```python
from build123d import *

# Parameters (mm, degrees)
SKETCH1_W           = 40
SKETCH1_H           = 15
BOSS_EXTRUDE1_DEPTH = 20
SKETCH2_W           = 35.032113562
SKETCH2_H           = 10.660333008
CUT_EXTRUDE1_DEPTH  = 10
SKETCH3_R           = 4
BOSS_EXTRUDE2_DEPTH = 35.032113562
SKETCH4_R           = 3.332307017
BOSS_EXTRUDE3_DEPTH = 10
BOSS_EXTRUDE4_START = 10
SKETCH5_R           = 3.332307017
BOSS_EXTRUDE4_DEPTH = 10
SCALE1_SCALE        = 0.7


with BuildPart() as part:
    # Sketch1 → Boss-Extrude1 (new body)
    with BuildSketch(Plane(origin=(0, 0, 0), x_dir=(1, 0, 0), z_dir=(0, 1, 0))):
        Rectangle(SKETCH1_W, SKETCH1_H)
    extrude(amount=BOSS_EXTRUDE1_DEPTH)

    # Sketch2 → Cut-Extrude1 (cut)
    with BuildSketch(Plane(origin=(0, 20, 0), x_dir=(1, 0, 0), z_dir=(0, 1, 0))):
        Rectangle(SKETCH2_W, SKETCH2_H)
    extrude(amount=-CUT_EXTRUDE1_DEPTH, mode=Mode.SUBTRACT)

    # Sketch3 → Boss-Extrude2 (add)
    with BuildSketch(Plane(origin=(-17.516056781, 0, 0), x_dir=(0, 0, -1), z_dir=(1, 0, 0))):
        with Locations((0, 10)):
            Circle(SKETCH3_R)
    extrude(amount=BOSS_EXTRUDE2_DEPTH)

    # Sketch4 → Boss-Extrude3 (add)
    with BuildSketch(Plane.ZY.offset(20)):
        with Locations((0, 10)):
            Circle(SKETCH4_R)
    extrude(amount=BOSS_EXTRUDE3_DEPTH)

    # Sketch5 → Boss-Extrude4 (add)
    with BuildSketch(Plane(origin=(20, 0, 0), x_dir=(0, 0, -1), z_dir=(1, 0, 0)).offset(BOSS_EXTRUDE4_START)):
        with Locations(Location((0, 10, 0), (0, 0, 180))):
            Circle(SKETCH5_R)
    extrude(amount=-BOSS_EXTRUDE4_DEPTH)


with BuildPart() as part_1:
    # Scale1: scaled about (0, 0, 0)
    add(part.part.scale(SCALE1_SCALE))


solid = part_1.part
```
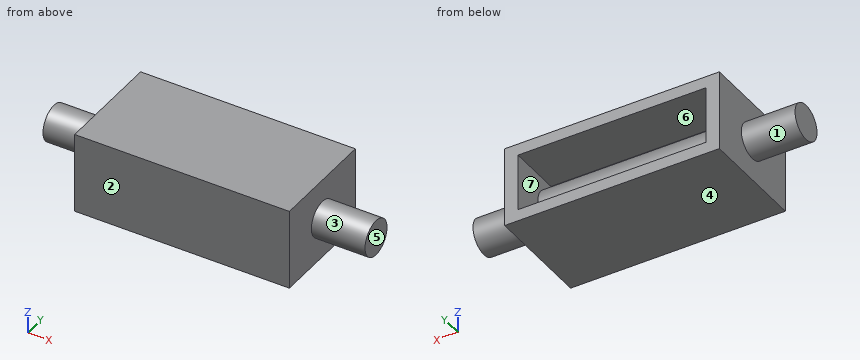
Check sheet for the modelled part. Datum: model origin and axes. Units: mm. Face numbers are marked on the shaded views. A direction names the side the tool comes from. Coordinates: 2 decimals unless noted, no trailing zeros. Order: outer loops, then holes, each group sorted by start corner. A loop starts at its lowest first (then second) coordinate and runs counter-clockwise, first axis right, second up. Notation, with made-up numbers: M 79.5,32.25 L 92.5,32.25 A23 cw 92.5,70.25 Z; hole C -25.75,59.25 d5. An arc over 180 degrees is marked long. One line per question, with ' | ' between items. Start each with the question number.
Item 1: Access from +Z, -Z, +X, -X, +Y, -Y to the whole of each face (thin tool, end or side, straight path). Record for the marked faces 1, 2 and 3.
Item 2: Sectioned sample at A-A on y = 13.25. Record the cut outline in (x, z), and give its area (3 significant figures).
Item 3: Material ranges on line 1 (X direction, y = 12.25, z = 2); line 2 (Z direction, x = -6, y = 10); line 3 (Z direction, x = -4, y = 7.25), recorded low to high.
Item 4: Sectioned sample at D-D on y = 3.25. Record the cut outline in (x, z), and give its area (3 significant figures).
Item 5: Sectioned sample at B-B on z = 0. Record the cut outline in (x, y), and give its area (3 significant figures).
Item 6: Mould release check, pull along X, two halves, no side actions. Record for the marked faces 4, 5, 6 and 7: pulls with the +X half, pulls with the -X half, needs draft (parallel to the pull), parting line crosses it, or undercut.
Item 7: Sectioned sample at C-C on x = -8. Record the cut outline in (y, z).
Answer below:
1) face 1: -X | face 2: +Z, -Z, +X, -X, -Y | face 3: +X
2) outline: M -14,-5.25 L 14,-5.25 L 14,5.25 L -14,5.25 Z; hole M -12.26,-3.73 L 12.26,-3.73 L 12.26,3.73 L -12.26,3.73 Z | area: 111 mm^2
3) line 1: x = -14 to -12.26, 12.26 to 14 | line 2: z = -5.25 to -3.73, 3.73 to 5.25 | line 3: z = -5.25 to -3.73, -2.79 to 2.79, 3.73 to 5.25
4) outline: M -14,-5.25 L 14,-5.25 L 14,5.25 L -14,5.25 Z | area: 294 mm^2
5) outline: M -21,4.67 L -14,4.67 L -14,0 L 14,0 L 14,4.67 L 21,4.67 L 21,9.33 L 14,9.33 L 14,14 L 12.26,14 L 12.26,9.8 L -12.26,9.8 L -12.26,14 L -14,14 L -14,9.33 L -21,9.33 Z | area: 354 mm^2
6) face 4: needs draft | face 5: pulls with the +X half | face 6: undercut | face 7: undercut
7) outline: M 0,-5.25 L 14,-5.25 L 14,-3.73 L 7,-3.73 L 7,-2.8 A2.8 ccw 7,2.8 L 7,3.73 L 14,3.73 L 14,5.25 L 0,5.25 Z
